```python
from build123d import *

# Parameters (mm, degrees)
SKETCH1_W           = 5
SKETCH1_H           = 53
SKETCH4_OUTSIDE_W   = 22.97
SKETCH4_OUTSIDE_H   = 22.97
SKETCH4_OUTSIDE_R   = 4
EXTRUDE1_DEPTH      = 4.5
SKETCH5_OUTSIDE_W   = 22.97
SKETCH5_OUTSIDE_H   = 22.97
SKETCH5_OUTSIDE_R   = 4
EXTRUDE2_DEPTH      = 4.5
EXTRUDE3_DEPTH      = 28.427176304
EXTRUDE3_DEPTH_BACK = 28.427176304
SKETCH6_W           = 7.231066263
SKETCH6_H           = 10
SKETCH6_W_2         = 2.606547141
CHAMFER1_SIZE       = 0.2


with BuildPart() as part:
    # Sketch1 → Revolve1 (revolve)
    with BuildSketch(Plane(origin=(0, 0, 0), x_dir=(0, 0, -1), z_dir=(1, 0, 0))):
        with Locations((-2.5, 0)):
            Rectangle(SKETCH1_W, SKETCH1_H)
    revolve(axis=Axis((0, 26.5, 0), (0, -1, 0)))

    # Sketch2 → M5 Tapped Hole1 (revolve, cut)
    with BuildSketch(Plane(origin=(0, 26.5, 0), x_dir=(0, 0, 1), z_dir=(1, 0, 0))):
        Polygon((0, 0), (0, 11.6618073), (2.1, 10.4), (2.1, 0), align=None)
    m5_tapped_hole1 = revolve(axis=Axis((0, 32.85, 0), (0, -1, 0)), mode=Mode.SUBTRACT)

    # Mirror1: M5 Tapped Hole1 across plane
    add(m5_tapped_hole1.mirror(Plane.ZX), mode=Mode.SUBTRACT)

    # Sketch4 outside → Extrude1 (cut)
    with BuildSketch(Plane.XZ.offset(26.5)):
        Rectangle(SKETCH4_OUTSIDE_W, SKETCH4_OUTSIDE_H)
        with Locations(Location((0, 0, 0), (0, 0, 270))):
            Circle(SKETCH4_OUTSIDE_R, mode=Mode.SUBTRACT)
    extrude(amount=-EXTRUDE1_DEPTH, mode=Mode.SUBTRACT)

    # Sketch5 outside → Extrude2 (cut)
    with BuildSketch(Plane(origin=(0, 26.5, 0), x_dir=(1, 0, 0), z_dir=(0, 1, 0))):
        Rectangle(SKETCH5_OUTSIDE_W, SKETCH5_OUTSIDE_H)
        with Locations(Location((0, 0, 0), (0, 0, 90))):
            Circle(SKETCH5_OUTSIDE_R, mode=Mode.SUBTRACT)
    extrude(amount=-EXTRUDE2_DEPTH, mode=Mode.SUBTRACT)

    # Sketch6 → Extrude3 (cut, two sides: drawn at the far end of the back side and taken through both)
    with BuildSketch(Plane(origin=(0, 0, 0), x_dir=(0, 0, -1), z_dir=(1, 0, 0)).offset(-EXTRUDE3_DEPTH_BACK)):
        with Locations((-7.615533132, 0)):
            Rectangle(SKETCH6_W, SKETCH6_H)
        with Locations((5.303273571, 0)):
            Rectangle(SKETCH6_W_2, SKETCH6_H)
    extrude(amount=EXTRUDE3_DEPTH + EXTRUDE3_DEPTH_BACK, mode=Mode.SUBTRACT)

    # Chamfer1
    chamfer1_edges = [part.edges().sort_by_distance(p)[0] for p in [
        (0, -26.5, 4),
        (0, 26.5, 4),
    ]]
    chamfer(chamfer1_edges, length=CHAMFER1_SIZE)


solid = part.part
```
Input: part model. Units: mm. Frame: model coordinates. A direction names the side the tool comes from. Coordinates: 2 decimals unless noted, no trailing zeros. Loops run counter-clockwise (first coordinate to the right, second up) from the corner with the lowest first, then second, coordinate; pieces in that order, holes last.
Q1. Contact query for flat-ended pins moving along their axis: pin 1 (3.5 mm diameter, centred on x = 0, z = 0, fed in from -Y); pin 2 (1 mm diameter, centred on y = 14.5, z = 3.5, fed in from -X); pin 3 (1.5 mm diameter, centred on x = 3.5, y = 20, fed in from +Z). Output: stop coordinate, or through.
Results are:
pin 1: stops at y = -15.89
pin 2: stops at x = -4
pin 3: stops at z = 4.18
Q2. Section B-B, the plane y = -20. Return the cut outline in (x, z), and give its area (3 significant figures).
Results are:
outline: circle Ø10 at (0, 0); hole circle Ø4.2 at (0, 0)
area: 64.7 mm2
Q3. Section A-A, the plane y = 11.5. Return the cut outline in (x, z), and give its area (3 significant figures).
Results are:
outline: circle Ø10 at (0, 0)
area: 78.5 mm2
Q4. Section C-C, the plane y = -3. Return the cut outline in (x, z), and give its area (3 significant figures).
Results are:
outline: (-3, -4) - (3, -4) arc R5 ccw to (3, 4) - (-3, 4) arc R5 ccw to start
area: 70.4 mm2
Q5. Set-up query: faces 1 (the cylindrical face through (-0.631, -21.373, 2.003)), 2 (the flat face through (0, 5, 4.4)), 3 (the cylindrical face through (-0.631, 21.373, 2.003)). Return all of +Z, -Z, +X, -X, +Y, -Y with unobstructed straight access to the full face (end or side cutting, diameter ignored); none if empty.
Results are:
face 1: -Y
face 2: +Z, +X, -X
face 3: +Y
Q6. Mould query, pull axis Z, two halves, no side actions, for faces 4 (the cylindrical face through (-3.379, 0.308, -3.685)), 5 (the conical face through (-0.11, 15.06, 0.35)), 6 (the flat face through (0, 0, -4)). Classes: +Z half, -Z half, draft (parallel to the pull), parting line (faces both ways), or undercut.
Results are:
face 4: parting line
face 5: undercut
face 6: -Z half
Q7. Line query: line 1 along X through (y, z) = (20.5, 0); line 2 along X through (y, z) = (23.5, 0). Output: solid intervals per line, ascending.
Results are:
line 1: x = -5 to -2.1, 2.1 to 5
line 2: x = -4 to -2.1, 2.1 to 4
